from build123d import *

# Parameters (mm, degrees)
BASE_BLOCK_PROFILE_SKETCH_W       = 96
BASE_BLOCK_PROFILE_SKETCH_H       = 35
BASE_BLOCK_DEPTH                  = 55
BASE_STEP_RECESS_DEPTH            = 81.956778592
BASE_STEP_RECESS_DEPTH_BACK       = 35
BASE_GROOVE_20X20_SKETCH_W        = 20
BASE_GROOVE_20X20_SKETCH_H        = 10
BASE_GROOVE_20X20_DEPTH           = 110
UPRIGHT_PAD_SKETCH_W              = 12
UPRIGHT_PAD_SKETCH_H              = 110
UPRIGHT_PAD_DEPTH                 = 15
LUG_PLATE_DEPTH                   = 12
LUG_START                         = 8
LUG_HUB_SKETCH_R                  = 22.5
LUG_HUB_DEPTH                     = 8
LUG_BORE_20_SKETCH_R              = 10
LUG_BORE_20_DEPTH                 = 20
SIDE_ARM_A_DEPTH                  = 16
SIDE_START                        = -16
SIDE_ARM_B_DEPTH                  = 16
ARM_B_EYE_HOLE_14_SKETCH_R        = 7
ARM_B_EYE_HOLE_14_DEPTH           = 16
ARM_START                         = -16
ARM_A_EYE_HOLE_14_SKETCH_R        = 7
ARM_A_EYE_HOLE_14_DEPTH           = 16
CROSS_WEB_SKETCH_W                = 16
CROSS_WEB_SKETCH_H                = 78
CROSS_WEB_DEPTH                   = 50
TRIANGULAR_RELIEF_CUT_REACH       = 156.306
COUNTERBORED_BOLT_HOLE_AT_2_COUNT = 2
COUNTERBORED_BOLT_HOLE_AT_2_PITCH = 35


with BuildPart() as part:
    # Base Block Profile Sketch → Base Block (new, symmetric)
    with BuildSketch(Plane.XY):
        with Locations((0, 17.5)):
            Rectangle(BASE_BLOCK_PROFILE_SKETCH_W, BASE_BLOCK_PROFILE_SKETCH_H)
    extrude(amount=BASE_BLOCK_DEPTH, both=True)

    # Base Step Recess Sketch → Base Step Recess (cut, two sides: drawn at the far end of the back side and taken through both)
    with BuildSketch(Plane(origin=(0, 35, 0), x_dir=(1, 0, 0), z_dir=(0, 1, 0)).offset(-BASE_STEP_RECESS_DEPTH_BACK)):
        Polygon((48, 55), (47.003525264, 55), (2, 55), (2, -55), (48, -55), align=None)
    extrude(amount=BASE_STEP_RECESS_DEPTH + BASE_STEP_RECESS_DEPTH_BACK, mode=Mode.SUBTRACT)

    # Base Groove 20x20 Sketch → Base Groove 20x20 (cut)
    with BuildSketch(Plane.XY.offset(55)):
        with Locations((-18, 5)):
            Rectangle(BASE_GROOVE_20X20_SKETCH_W, BASE_GROOVE_20X20_SKETCH_H)
    extrude(amount=-BASE_GROOVE_20X20_DEPTH, mode=Mode.SUBTRACT)

    # Upright Pad Sketch → Upright Pad (add)
    with BuildSketch(Plane(origin=(0, 35, 0), x_dir=(1, 0, 0), z_dir=(0, 1, 0))):
        with Locations((-4, 0)):
            Rectangle(UPRIGHT_PAD_SKETCH_W, UPRIGHT_PAD_SKETCH_H)
    extrude(amount=UPRIGHT_PAD_DEPTH)

    # Lug Plate Sketch → Lug Plate (add)
    with BuildSketch(Plane(origin=(2, 0, 0), x_dir=(0, 0, -1), z_dir=(1, 0, 0))):
        with BuildLine():
            Line((-35, 50), (-21.299956881, 90.249954267))
            ThreePointArc((-21.299956881, 90.249954267), (0, 105.5), (21.299956881, 90.249954267))
            Line((21.299956881, 90.249954267), (35, 50))
            Line((35, 50), (0, 50))
            Line((0, 50), (-35, 50))
        make_face()
    extrude(amount=-LUG_PLATE_DEPTH)

    # Lug Hub Sketch → Lug Hub (add)
    with BuildSketch(Plane(origin=(2, 0, 0), x_dir=(0, 0, -1), z_dir=(1, 0, 0)).offset(LUG_START)):
        with Locations(Location((0, 83, 0), (0, 0, 90))):
            Circle(LUG_HUB_SKETCH_R)
    extrude(amount=-LUG_HUB_DEPTH)

    # Lug Bore Ø20 Sketch → Lug Bore Ø20 (cut)
    with BuildSketch(Plane(origin=(10, 0, 0), x_dir=(0, 0, -1), z_dir=(1, 0, 0))):
        with Locations(Location((0, 83, 0), (0, 0, 90))):
            Circle(LUG_BORE_20_SKETCH_R)
    extrude(amount=-LUG_BORE_20_DEPTH, mode=Mode.SUBTRACT)

    # Side Arm A Sketch → Side Arm A (add)
    with BuildSketch(Plane(origin=(0, 0, -55), x_dir=(-1, 0, 0), z_dir=(0, 0, -1))):
        with BuildLine():
            Line((8, 0), (-48, 0))
            ThreePointArc((-48, 0), (-61.689486066, 11.067770261), (-53.734388308, 26.771718394))
            Line((-53.734388308, 26.771718394), (-2, 50))
            Line((-2, 50), (10, 50))
            Line((10, 50), (10, 35))
            Line((10, 35), (10, 10))
            Line((10, 10), (8, 10))
            Line((8, 10), (8, 0))
        make_face()
    extrude(amount=-SIDE_ARM_A_DEPTH)

    # Side Arm B Sketch → Side Arm B (add)
    with BuildSketch(Plane.XY.offset(55).offset(SIDE_START)):
        with BuildLine():
            Line((-8, 0), (48, 0))
            ThreePointArc((48, 0), (61.689486066, 11.067770261), (53.734388308, 26.771718394))
            Line((53.734388308, 26.771718394), (2, 50))
            Line((2, 50), (-10, 50))
            Line((-10, 50), (-10, 35))
            Line((-10, 35), (-13.136025353, 35))
            Line((-13.136025353, 35), (-13.136025353, 10))
            Line((-13.136025353, 10), (-8, 10))
            Line((-8, 10), (-8, 0))
        make_face()
    extrude(amount=SIDE_ARM_B_DEPTH)

    # Arm B Eye Hole Ø14 Sketch → Arm B Eye Hole Ø14 (cut)
    with BuildSketch(Plane.XY.offset(55)):
        with Locations((48, 14)):
            Circle(ARM_B_EYE_HOLE_14_SKETCH_R)
    extrude(amount=-ARM_B_EYE_HOLE_14_DEPTH, mode=Mode.SUBTRACT)

    # Arm A Eye Hole Ø14 Sketch → Arm A Eye Hole Ø14 (cut)
    with BuildSketch(Plane(origin=(0, 0, -55), x_dir=(-1, 0, 0), z_dir=(0, 0, -1)).offset(ARM_START)):
        with Locations(Location((-48, 14, 0), (0, 0, 180))):
            Circle(ARM_A_EYE_HOLE_14_SKETCH_R)
    extrude(amount=ARM_A_EYE_HOLE_14_DEPTH, mode=Mode.SUBTRACT)

    # Cross Web Sketch → Cross Web (add)
    with BuildSketch(Plane(origin=(0, 50, 0), x_dir=(1, 0, 0), z_dir=(0, 1, 0))):
        with Locations((10, 0)):
            Rectangle(CROSS_WEB_SKETCH_W, CROSS_WEB_SKETCH_H)
    extrude(amount=-CROSS_WEB_DEPTH)

    # Triangular Relief Sketch → Triangular Relief Cut (cut, up to next)
    with BuildSketch(Plane.XY.offset(39), mode=Mode.PRIVATE) as triangular_relief_cut_sk1:
        Polygon((2, 50), (18, 42.816141877), (18, 50), align=None)
    triangular_relief_cut_tool1 = extrude(triangular_relief_cut_sk1.sketch, amount=-TRIANGULAR_RELIEF_CUT_REACH, mode=Mode.PRIVATE) & part.part
    add(triangular_relief_cut_tool1.solids().sort_by_distance((12.666667, 47.605381, 39))[0], mode=Mode.SUBTRACT)

    # Sketch42 → Counterbored Bolt Hole (revolve, cut)
    with BuildSketch(Plane(origin=(-29, 35, 35), x_dir=(0, 0, 1), z_dir=(1, 0, 0))):
        Polygon((0, 0), (0, 35), (12, 35), (12, 6), (6, 6), (6, 0.145), (6.145, 0), align=None)
    counterbored_bolt_hole = revolve(axis=Axis((-29, 41.35, 35), (0, -1, 0)), mode=Mode.SUBTRACT)

    # Counterbored Bolt Hole at 2: Counterbored Bolt Hole ×2
    with Locations(*[(0, 0, -i * COUNTERBORED_BOLT_HOLE_AT_2_PITCH) for i in range(1, COUNTERBORED_BOLT_HOLE_AT_2_COUNT)]):
        add(counterbored_bolt_hole, mode=Mode.SUBTRACT)


solid = part.part
The model under review builds one solid part; all positions refer to its coordinate system, in mm. A direction names the side the tool comes from. Round coordinates to 2 decimals unless told otherwise and drop trailing zeros. Loops run counter-clockwise (first coordinate to the right, second up) from the corner with the lowest first, then second, coordinate; pieces in that order, holes last. Notation, with made-up numbers: M -18,11.25 L 5,11.25 A8 cw 5,18.25 Z; hole C 42.25,42 d6. An arc over 180 degrees is marked long. Answer as CSV lines item,"result".
1. We need section A-A (y = 14). Give the boundary of the cut face in (x, z).
Outcome:
outline,"M -48,-55 L 41,-55 L 41,-39 L 18,-39 L 18,39 L 41,39 L 41,55 L -48,55 Z; M 55,-55 L 62,-55 L 62,-39 L 55,-39 Z; M 55,39 L 62,39 L 62,55 L 55,55 Z; hole C -29,0 d24; hole C -29,35 d24"
2. Draft analysis for pull direction Y (two halves, no side actions). For faces 4 (the face through (61.63, 10.81, 46.89)), 5 (the face through (10, 88, -10)), 6 (the face through (2, 56, 0)), state which applies: pulls with the +Y half, pulls with the -Y half, needs draft (parallel to the pull), parting line crosses it, or undercut.
Outcome:
face 4,"parting line crosses it"
face 5,"needs draft"
face 6,"undercut"
3. For faces 1 (the face through (-28, 5, -33)), 2 (the face through (35, 17, 39)), 3 (the face through (-4, 50, 45)), list the 3-axis set-ups (+Z, -Z, +X, -X, +Y, -Y) from which the entire face can be reached by the end or side of a thin tool; tool diameter is ignored.
Outcome:
face 1,"+Z, -Z, -Y"
face 2,"+X, +Y, -Y"
face 3,"+Z, +X, -X, +Y"
4. We need section B-B (z = 0). Give the boundary of the cut face in (x, y) (3 decimals).
Outcome:
outline,"M -48,0 L -41,0 L -41,29 L -35,29 L -35,34.855 L -35.145,35 L -48,35 Z; M -23,29 L -17,29 L -17,10 L -8,10 L -8,0 L 18,0 L 18,42.816 L 2,50 L 2,60.5 L 10,60.5 L 10,73 L -10,73 L -10,35 L -22.855,35 L -23,34.855 Z; M -10,93 L 10,93 L 10,105.5 L -10,105.5 Z"
5. We need section C-C (x = 20). Give the boundary of the cut face in (y, z), plus the area to 3 significant figures.
Outcome:
outline,"M 0,-55 L 41.92,-55 L 41.92,-39 L 0,-39 Z; M 0,39 L 41.92,39 L 41.92,55 L 0,55 Z"
area,"1,340 mm2"
6. To check wall thickness, follow L1, parallel to Z at x = -29, y = 31; L2, parallel to X at y = 31, z = 0; L3, parallel to Z at x = -29, y = 12.5. State the ranges of each line that lie inside material, in increasing order. Write a range as [from, to].
Outcome:
L1,"z = [-55, -6], [6, 29], [41, 55]"
L2,"x = [-48, -35], [-23, 18]"
L3,"z = [-55, -12], [12, 23], [47, 55]"
7. Insertion check: pin 1 Ø15.5 at (x, z) = (-29, 35) entering from +Y; pin 2 Ø14 at (x, z) = (-29, 0) entering from -Y; pin 3 Ø3 at (y, z) = (37.5, -5) entering from +X. Each pin has a flat end and moves straight along its axis. Give the tip position at first contact, or say it passes through.
Outcome:
pin 1,"stops at y = 35"
pin 2,"stops at y = 29"
pin 3,"stops at x = 18"
8. We need section D-D (y = 83). Give the boundary of the cut face in (x, z), plus the area to 3 significant figures.
Outcome:
outline,"M -10,-23.77 L 2,-23.77 L 2,-22.5 L 10,-22.5 L 10,-10 L -10,-10 Z; M -10,10 L 10,10 L 10,22.5 L 2,22.5 L 2,23.77 L -10,23.77 Z"
area,"530 mm2"
